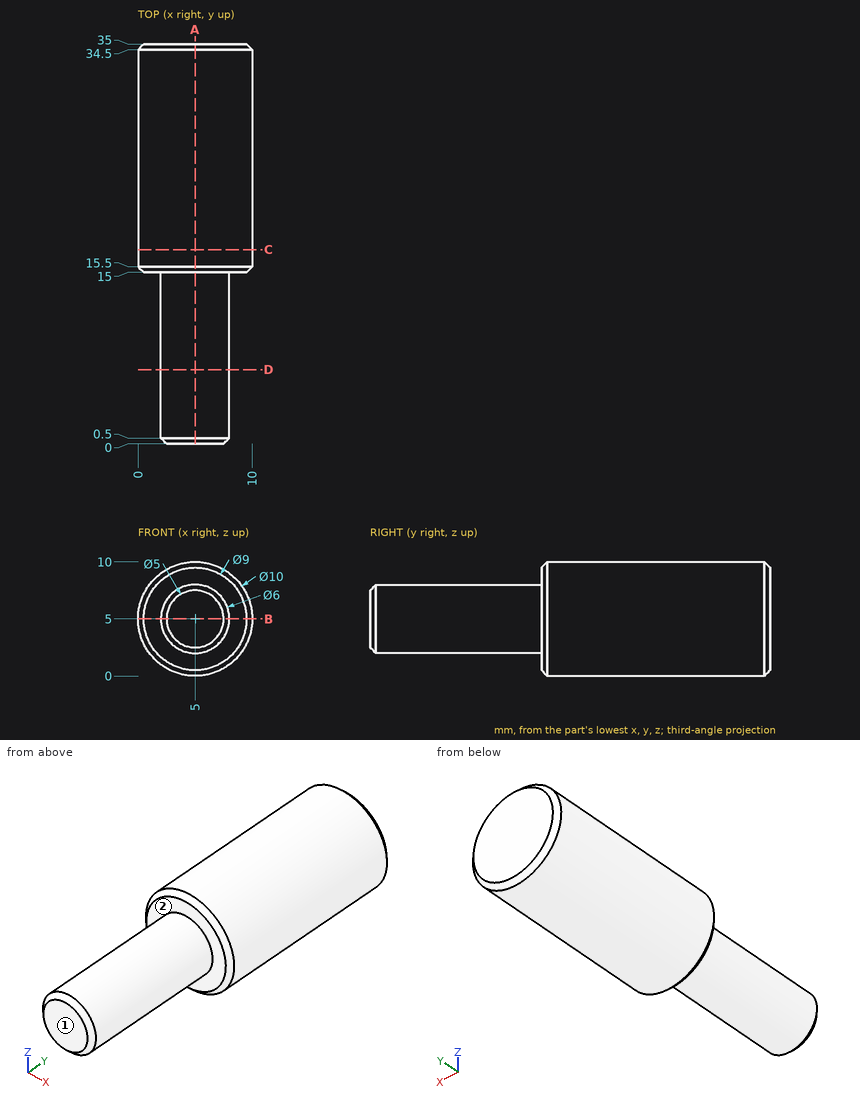
Print and shaded views of the part. All mm, measured from the part's lowest x, y and z. A direction names the side the tool comes from. Coordinates: 2 decimals unless noted, no trailing zeros. Order: outer loops, then holes, each group sorted by start corner. A loop starts at its lowest first (then second) coordinate and runs counter-clockwise, first axis right, second up. Notation, with made-up numbers: M -10.75,75 L 22.25,75 A25 cw 22.25,94 Z; hole C 14,79.25 d6. An arc over 180 degrees is marked long. One line per question, with ' | ' between items. Start each with the question number.
Q1. 3-axis set-ups, long thin cutter, end or side, ignore diameter. For the marked faces 1 and 2: which of +Z, -Z, +X, -X, +Y, -Y reach the whole face in a straight line?
Q2. Saw through at A-A (x = 5). List the corners of the cut face in (y, z), then the cut area to 3 significant figures.
Q3. Saw through at D-D (y = 6.5). List the corners of the cut face in (x, z), then the cut area to 3 significant figures.
Q4. Probe L1, parallel to X at y = 21.5, z = 5.25; L2, parallel to Y at x = 2.75, z = 1.5; L3, parallel to Z at x = 6.5, y = 5. List the from-to ranges inside material, lowest first. Write a range as from..to.
Q5. Flat gauge pins, fed straight in: pin 1 Ø1.5 at (y, z) = (12.5, 5.5) entering from +X; pin 2 Ø4 at (x, y) = (2, 7.5) entering from +Z; pin 3 Ø1 at (x, z) = (1, 8.5) entering from -Y. Where does each tip first touch, or does it go through?
Q6. Saw through at C-C (y = 17). List the corners of the cut face in (x, z).
Q7. Saw through at B-B (z = 5). List the corners of the cut face in (x, y), then the cut area to 3 significant figures.
Check values:
1) face 1: +Z, -Z, +X, -X, -Y | face 2: -Y
2) outline: M 0,2.5 L 0.5,2 L 15,2 L 15,0.5 L 15.5,0 L 34.5,0 L 35,0.5 L 35,9.5 L 34.5,10 L 15.5,10 L 15,9.5 L 15,8 L 0.5,8 L 0,7.5 Z | area: 289 mm2
3) outline: C 5,5 d6 | area: 28.3 mm2
4) L1: x = 0.01..9.99 | L2: y = 15..35 | L3: z = 2.4..7.6
5) pin 1: stops at x = 8 | pin 2: stops at z = 7.83 | pin 3: stops at y = 15.32
6) outline: C 5,5 d10
7) outline: M 0,15.5 L 0.5,15 L 2,15 L 2,0.5 L 2.5,0 L 7.5,0 L 8,0.5 L 8,15 L 9.5,15 L 10,15.5 L 10,34.5 L 9.5,35 L 0.5,35 L 0,34.5 Z | area: 289 mm2
